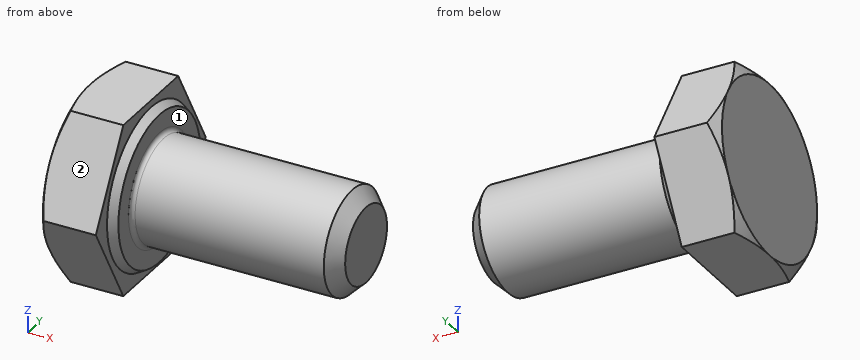
```python
from build123d import *

# Parameters (mm, degrees)
BASE_EXTRUDE_DEPTH = 4
CHAMFER_2_SIZE     = 0.8


with BuildPart() as part:
    # Sketch1 → Base-extrude (new body)
    with BuildSketch(Plane(origin=(0, 0, 0), x_dir=(0, 0, -1), z_dir=(1, 0, 0))):
        Polygon((5, 2.886751346), (5, -2.886751346), (0, -5.773502692), (-5, -2.886751346), (-5, 2.886751346), (0, 5.773502692), align=None)
    extrude(amount=BASE_EXTRUDE_DEPTH)

    # Sketch2 → Boss-Revolve1 (revolve)
    with BuildSketch(Plane.XY, mode=Mode.PRIVATE) as boss_revolve1_sk:
        Polygon((0, 0), (16, 0), (16, 2.134), (16, 3), (4, 3), (0, 3), align=None)
    revolve(boss_revolve1_sk.sketch.rotate(Axis((0, 0, 0), (-1, 0, 0)), 90), axis=Axis((0, 0, 0), (-1, 0, 0)))

    # Sketch3 → Cut-Revolve1 (revolve, cut)
    with BuildSketch(Plane.XY):
        Polygon((0, 5), (3.333333333, 10.773502692), (3.333333333, 15.773502692), (-10, 15.773502692), (-10, 5), align=None)
    revolve(axis=Axis((0, 0, 0), (1, 0, 0)), mode=Mode.SUBTRACT)

    # Sketch5 → Cut-Revolve2 (revolve, cut)
    with BuildSketch(Plane.XY):
        Polygon((4, 5), (0.666666667, 10.773502692), (0.666666667, 15.773502692), (10.666666667, 15.773502692), (10.666666667, 5), align=None)
    revolve(axis=Axis((0, 0, 0), (1, 0, 0)), mode=Mode.SUBTRACT)

    # Sketch4 → Cut-Revolve3 (revolve, cut)
    with BuildSketch(Plane.XY, mode=Mode.PRIVATE) as cut_revolve3_sk:
        Polygon((4, 4.312264973), (3.5, 4.600940108), (3.5, 15.773502692), (4, 15.773502692), align=None)
    revolve(cut_revolve3_sk.sketch.rotate(Axis((0, 0, 0), (1, 0, 0)), 90), axis=Axis((0, 0, 0), (1, 0, 0)), mode=Mode.SUBTRACT)

    # Chamfer 2
    chamfer_2_edges = [part.edges().sort_by_distance(p)[0] for p in [
        (16, 0, 3),
    ]]
    chamfer(chamfer_2_edges, length=CHAMFER_2_SIZE)

    # Sketch9 → Revolve1 (revolve)
    with BuildSketch(Plane.XY, mode=Mode.PRIVATE) as revolve1_sk:
        with BuildLine():
            Line((4, 3.25), (4, 3))
            Line((4, 3), (4.25, 3))
            ThreePointArc((4.25, 3), (4.073223305, 3.073223305), (4, 3.25))
        make_face()
    revolve(revolve1_sk.sketch.rotate(Axis((0, 0, 0), (1, 0, 0)), 90), axis=Axis((0, 0, 0), (1, 0, 0)))


solid = part.part
```
Work out the finished part from the listing and answer in its coordinate system (mm). Face numbers are marked on the shaded views. A direction names the side the tool comes from. Round coordinates to 2 decimals unless told otherwise and drop trailing zeros. Write each loop counter-clockwise with the first axis right and the second up, starting at its lowest first coordinate (ties: lowest second). Pieces come first, ordered by that corner, then holes. Notation, with made-up numbers: (-8.75, 20.25) -> (44.25, 20.25) arc R26 ccw to (44.25, 40.25) -> close; hole circle Ø4 at (58.5, 37). An arc over 180 degrees is marked (long way). Write each question's results on one line, items separated by ' | '.
Q1. Straight lines are drawn through the part: line 1 along X through (y, z) = (-4.5, -1.5); line 2 along X through (y, z) = (3, -1.75); line 3 along Z through (x, y) = (9.5, -2.25). For each, find the intervals that lie inside material, in ascending order. Write a range as [from, to].
Data:
line 1: [0, 3.5] | line 2: [0, 4] | line 3: [-1.98, 1.98]
Q2. Section A-A, the plane x = 8.75 is taken. Write down the section's boundary in (y, z), then the cut area to 3 significant figures.
Data:
outline: circle Ø6 at (0, 0) | area: 28.3 mm^2
Q3. Flat-ended cylindrical pins translate along their axes: P1, Ø4, axis at x = 13.5, z = 3, coming from the -Y side; P2, Ø6, axis at x = 10.5, y = 4.5, coming from the +Z side; P3, Ø2, axis at x = 11, y = -4.5, coming from the -Z side; P4, Ø1, axis at x = 6.5, z = 2, coming from the -Y side. Find the tip coordinate at first contact, or state that the pin passes through.
Data:
P1: y = -2.83 | P2: z = 2.6 | P3: through | P4: y = -2.6
Q4. Which of the six approach directions +Z, -Z, +X, -X, +Y, -Y give full straight-line access (tool end or side, diameter ignored) to the marked faces 1 and 2?
Data:
face 1: +X | face 2: +Z, +X, -X, -Y
